```python
from build123d import *

# Parameters (mm, degrees)
SKETCH_1_W          = 55
SKETCH_1_H          = 100
EXTRUDE_1_DEPTH     = 12
SKETCH_2_W          = 50
SKETCH_2_H          = 100
CUT_EXTRUDE_1_DEPTH = 1.5


with BuildPart() as part:
    # 草图1 → 凸台-拉伸1 (new body)
    with BuildSketch(Plane.XY):
        Rectangle(SKETCH_1_W, SKETCH_1_H)
    extrude(amount=EXTRUDE_1_DEPTH)

    # 草图2 → 切除-拉伸1 (cut)
    with BuildSketch(Plane.XY.offset(12)):
        Rectangle(SKETCH_2_W, SKETCH_2_H)
    extrude(amount=-CUT_EXTRUDE_1_DEPTH, mode=Mode.SUBTRACT)


solid = part.part
```
Work out the finished part from the listing and answer in its coordinate system (mm). Coordinates: 2 decimals unless noted, no trailing zeros. Write each loop counter-clockwise with the first axis right and the second up, starting at its lowest first coordinate (ties: lowest second). Pieces come first, ordered by that corner, then holes.
Q1. Find the intervals of material crossed by line 1 (Z direction, x = -10, y = -27); line 2 (X direction, y = 4.5, z = 11), in increasing order.
Q2. This flat-tipped pin is pushed along its axis until it touches: pin 1 Ø1.5 at (x, y) = (5, -16) entering from +Z. Where does it stop, or does it pass through?
Q3. A cutting plane is placed at B-B, the plane x = 17.5. Give the vertices of the cut face in (y, z), then the cut area to 3 significant figures.
Q4. Determine the mould class of faces 1 (the face through (-27.5, -1, 6)), 2 (the face through (27.5, -1, 6)), 3 (the face through (26, 1, 12)), 4 (the face through (0, 1, 10.5)) for opening direction X: released by +X, released by -X, zero draft, split by the parting line, or undercut.
Q5. A cutting plane is placed at A-A, the plane y = -24. Give the vertices of the cut face in (x, z), then the cut area to 3 significant figures.
Findings below:
1. line 1: z = 0 to 10.5
1. line 2: x = -27.5 to -25, 25 to 27.5
2. pin 1: stops at z = 10.5
3. outline: (-50, 0) - (50, 0) - (50, 10.5) - (-50, 10.5) - close
3. area: 1,050 mm2
4. face 1: released by -X
4. face 2: released by +X
4. face 3: zero draft
4. face 4: undercut
5. outline: (-27.5, 0) - (27.5, 0) - (27.5, 12) - (25, 12) - (25, 10.5) - (-25, 10.5) - (-25, 12) - (-27.5, 12) - close
5. area: 585 mm2
